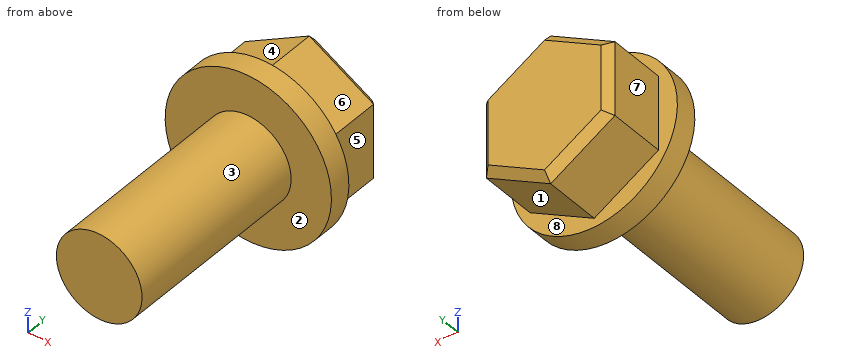
from build123d import *

# Parameters (mm, degrees)
SHANK_SKETCH_12_7_R         = 6.35
SHANK_12_7_DEPTH            = 28.19
FLANGE_SKETCH_24_64_R       = 12.32
FLANGE_24_64_DEPTH          = 3.3
HEX_HEAD_DEPTH              = 9.4
EDGE_CHAMFER_1_16X45_A_SIZE = 1.16
EDGE_CHAMFER_1_16X45_B_SIZE = 1.16
EDGE_CHAMFER_1_16X45_C_SIZE = 1.16


with BuildPart() as part:
    # Shank Sketch Ø12.7 → Shank Ø12.7 (new body)
    with BuildSketch(Plane(origin=(0, 0, 0), x_dir=(1, 0, 0), z_dir=(0, 1, 0))):
        with Locations(Location((0, 0, 0), (0, 0, 90))):
            Circle(SHANK_SKETCH_12_7_R)
    extrude(amount=SHANK_12_7_DEPTH)

    # Flange Sketch Ø24.64 → Flange Ø24.64 (add)
    with BuildSketch(Plane(origin=(0, 28.19, 0), x_dir=(1, 0, 0), z_dir=(0, 1, 0))):
        with Locations(Location((0, 0, 0), (0, 0, 270))):
            Circle(FLANGE_SKETCH_24_64_R)
    extrude(amount=FLANGE_24_64_DEPTH)

    # Hex Head Sketch → Hex Head (add)
    with BuildSketch(Plane(origin=(0, 31.49, 0), x_dir=(1, 0, 0), z_dir=(0, 1, 0))):
        Polygon((0, 11), (-9.526279442, 5.5), (-9.526279442, -5.5), (0, -11), (9.526279442, -5.5), (9.526279442, 5.5), align=None)
    extrude(amount=HEX_HEAD_DEPTH)

    # Edge Chamfer 1.16x45 A
    edge_chamfer_1_16x45_a_edges = [part.edges().sort_by_distance(p)[0] for p in [
        (-9.526279442, 40.89, 0),
        (-4.763139721, 40.89, 8.25),
    ]]
    chamfer(edge_chamfer_1_16x45_a_edges, length=EDGE_CHAMFER_1_16X45_A_SIZE)

    # Edge Chamfer 1.16x45 B
    edge_chamfer_1_16x45_b_edges = [part.edges().sort_by_distance(p)[0] for p in [
        (4.763139721, 40.89, -8.25),
        (9.526279442, 40.89, 0),
        (5.343139721, 40.89, 7.915136844),
    ]]
    chamfer(edge_chamfer_1_16x45_b_edges, length=EDGE_CHAMFER_1_16X45_B_SIZE)

    # Edge Chamfer 1.16x45 C
    edge_chamfer_1_16x45_c_edges = [part.edges().sort_by_distance(p)[0] for p in [
        (-4.763139721, 40.89, -8.25),
    ]]
    chamfer(edge_chamfer_1_16x45_c_edges, length=EDGE_CHAMFER_1_16X45_C_SIZE)


solid = part.part
Geometry: final body of the model. Coordinates: model frame, mm. Face numbers are marked on the shaded views. A direction names the side the tool comes from. Round coordinates to 2 decimals unless told otherwise and drop trailing zeros. Loops run counter-clockwise (first coordinate to the right, second up) from the corner with the lowest first, then second, coordinate; pieces in that order, holes last. Notation, with made-up numbers: (14.5, -27) -> (27.5, -27) arc R29 ccw to (27.5, -1) -> close; hole circle Ø7 at (45.5, 36.25). An arc over 180 degrees is marked (long way). One line per question, with ' | ' between items. Start each with the question number.
1. Set-up query: the marked faces 4, 5, 6, 7 and 8. Return all of +Z, -Z, +X, -X, +Y, -Y with unobstructed straight access to the full face (end or side cutting, diameter ignored); none if empty.
2. Section B-B on y = 36.5. Output: boundary loops of the cut face in (x, z).
3. Section C-C on z = -2.5. Output: boundary loops of the cut face in (x, y), and give its area (3 significant figures).
4. Mould query, pull axis Z, two halves, no side actions, for the marked faces 1, 2 and 3. Classes: pulls with the +Z half, pulls with the -Z half, needs draft (parallel to the pull), parting line crosses it, or undercut.
5. Section A-A on z = 0. Output: boundary loops of the cut face in (x, y), and give its area (3 significant figures).
6. Section D-D on x = 10. Output: boundary loops of the cut face in (y, z), and give its area (3 significant figures).
7. Contact query for flat-ended pins moving along their axis: pin 1 (6.5 mm diameter, centred on y = 36.5, z = 2, fed in from -X); pin 2 (6 mm diameter, centred on x = 9.5, y = 36.5, fed in from +Z); pin 3 (1 mm diameter, centred on x = 6, z = -4, fed in from -Y). Output: stop coordinate, or through.
8. Line query: line 1 along Y through (x, z) = (10, -6); line 2 along Z through (x, y) = (0.25, 27); line 3 along Y through (x, z) = (-7, -3.5). Output: solid intervals per line, ascending. Write a range as [from, to].
Returned:
1) face 4: +Z, -X, +Y | face 5: +Z, -Z, +X, +Y | face 6: +Z, +X, +Y | face 7: +Z, -Z, -X, +Y | face 8: +Y
2) outline: (-9.53, -5.5) -> (0, -11) -> (9.53, -5.5) -> (9.53, 5.5) -> (0, 11) -> (-9.53, 5.5) -> close
3) outline: (-12.06, 28.19) -> (-5.84, 28.19) -> (-5.84, 0) -> (5.84, 0) -> (5.84, 28.19) -> (12.06, 28.19) -> (12.06, 31.49) -> (9.53, 31.49) -> (9.53, 39.73) -> (8.37, 40.89) -> (-8.37, 40.89) -> (-9.53, 39.73) -> (-9.53, 31.49) -> (-12.06, 31.49) -> close | area: 586 mm2
4) face 1: pulls with the -Z half | face 2: needs draft | face 3: parting line crosses it
5) outline: (-12.32, 28.19) -> (-6.35, 28.19) -> (-6.35, 0) -> (6.35, 0) -> (6.35, 28.19) -> (12.32, 28.19) -> (12.32, 31.49) -> (9.53, 31.49) -> (9.53, 39.73) -> (8.37, 40.89) -> (-8.37, 40.89) -> (-9.53, 39.73) -> (-9.53, 31.49) -> (-12.32, 31.49) -> close | area: 617 mm2
6) outline: (28.19, -7.2) -> (31.49, -7.2) -> (31.49, 7.2) -> (28.19, 7.2) -> close | area: 47.5 mm2
7) pin 1: stops at x = -9.53 | pin 2: stops at z = 7.25 | pin 3: stops at y = 28.19
8) line 1: y = [28.19, 31.49] | line 2: z = [-6.35, 6.35] | line 3: y = [28.19, 40.89]
